Geometry: see drawing. Coordinates: mm, zero at the bounding-box minimum. Coordinates: 2 decimals unless noted, no trailing zeros. Order: outer loops, then holes, each group sorted by start corner. A loop starts at its lowest first (then second) coordinate and runs counter-clockwise, first axis right, second up. Notation, with made-up numbers: M 60.5,87.25 L 97.5,87.25 A31 cw 97.5,116.25 Z; hole C 68,10 d3. An arc over 180 degrees is marked long. Answer in a Markdown table with one row per item.
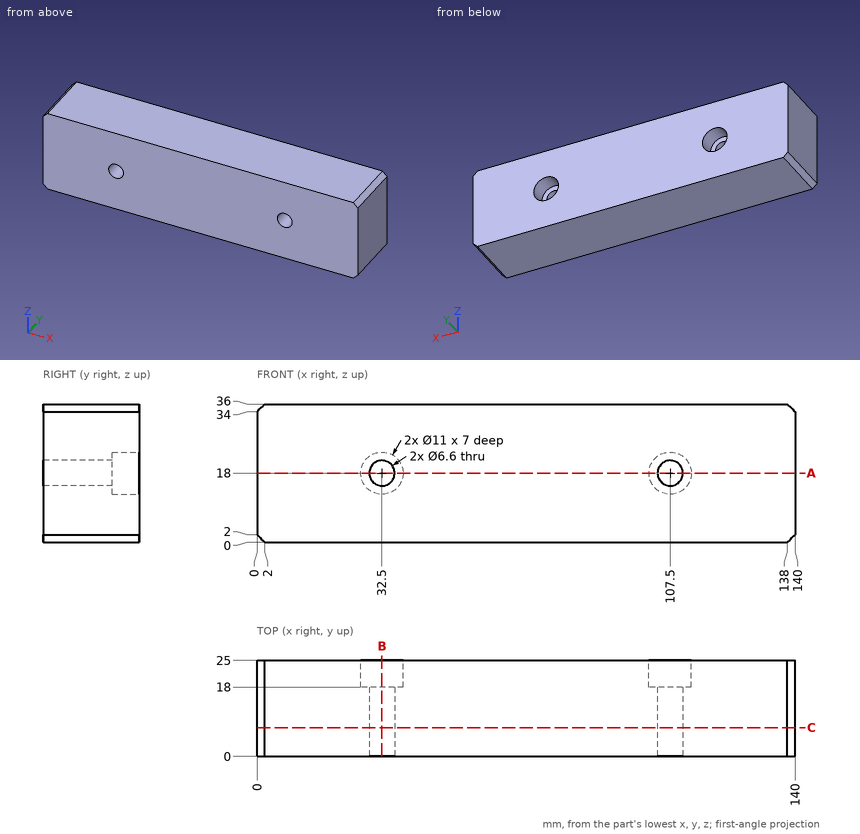
1) Contact query for flat-ended pins moving along their axis: pin 1 (6.5 mm diameter, centred on x = 32.5, z = 18, fed in from +Y); pin 2 (3.5 mm diameter, centred on x = 107.5, z = 20.5, fed in from +Y). Output: stop coordinate, or through.
Resolved:
| item | result |
|---|---|
| pin 1 | passes through |
| pin 2 | stops at y = 18 |
2) Cut plane C-C, the plane y = 7.5. Output: boundary loops of the cut face in (x, z), and give its area (3 significant figures).
Resolved:
| item | result |
|---|---|
| outline | M 0,2 L 2,0 L 138,0 L 140,2 L 140,34 L 138,36 L 2,36 L 0,34 Z; hole C 32.5,18 d6.6; hole C 107.5,18 d6.6 |
| area | 4,960 mm2 |
3) Cut plane A-A, the plane z = 18. Output: boundary loops of the cut face in (x, y).
Resolved:
| item | result |
|---|---|
| outline | M 0,0 L 29.2,0 L 29.2,18 L 27,18 L 27,25 L 0,25 Z; M 35.8,0 L 104.2,0 L 104.2,18 L 102,18 L 102,25 L 38,25 L 38,18 L 35.8,18 Z; M 110.8,0 L 140,0 L 140,25 L 113,25 L 113,18 L 110.8,18 Z |
4) Material intervals for probe 1 along X at (y, z) = (20.25, 18); probe 2 along X at (y, z) = (4.25, 18); probe 3 along Z at (x, y) = (107.5, 6.75), sorted ascending.
Resolved:
| item | result |
|---|---|
| probe 1 | x = 0 to 27, 38 to 102, 113 to 140 |
| probe 2 | x = 0 to 29.2, 35.8 to 104.2, 110.8 to 140 |
| probe 3 | z = 0 to 14.7, 21.3 to 36 |
5) Cut plane B-B, the plane x = 32.5. Output: boundary loops of the cut face in (y, z), and give its area (3 significant figures).
Resolved:
| item | result |
|---|---|
| outline | M 0,0 L 25,0 L 25,12.5 L 18,12.5 L 18,14.7 L 0,14.7 Z; M 0,21.3 L 18,21.3 L 18,23.5 L 25,23.5 L 25,36 L 0,36 Z |
| area | 704 mm2 |
